Here's how the part is built. I have some questions about the finished solid (model axes, mm). Face numbers are marked on the shaded views. A direction names the side the tool comes from. Coordinates: 2 decimals unless noted, no trailing zeros. Order: outer loops, then holes, each group sorted by start corner. A loop starts at its lowest first (then second) coordinate and runs counter-clockwise, first axis right, second up. Notation, with made-up numbers: M 0.25,39 L 30.25,39 A24 ccw 30.25,71 Z; hole C 0,42.25 d2. An arc over 180 degrees is marked long. One line per question, with ' | ' between items. Start each with the question number.
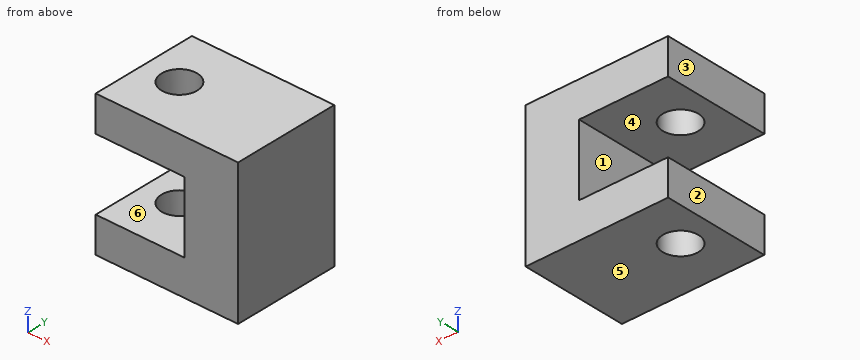
```python
from build123d import *

# Parameters (mm, degrees)
BOSS_EXTRUDE1_DEPTH = 30
SKETCH2_R           = 5
CUT_EXTRUDE1_DEPTH  = 54.851648071


with BuildPart() as part:
    # Sketch1 → Boss-Extrude1 (new body)
    with BuildSketch(Plane(origin=(0, 0, 0), x_dir=(1, 0, 0), z_dir=(0, 1, 0))):
        Polygon((-20, 10), (-20, 20), (20, 20), (20, -20), (-20, -20), (-20, -10), (5, -10), (5, 10), align=None)
    extrude(amount=BOSS_EXTRUDE1_DEPTH)

    # Sketch2 → Cut-Extrude1 (cut, through all)
    with BuildSketch(Plane(origin=(0, 0, -20), x_dir=(-1, 0, 0), z_dir=(0, 0, -1))):
        with Locations((10, 15)):
            Circle(SKETCH2_R)
    extrude(amount=-CUT_EXTRUDE1_DEPTH, mode=Mode.SUBTRACT)


solid = part.part
```
1. I need wall thicknesses on line 1 (Z direction, x = -4, y = 11.75); line 2 (Y direction, x = -10, z = -13.75); line 3 (X direction, y = 25, z = -4). Which ranges of each line are inside material? Lowest first, please.
2. We'd pull the mould along Z, two halves only. Please class the marked faces 3, 4, 5 and 6: released by +Z, released by -Z, zero draft, split by the parting line, or undercut.
3. Imagine slicing it at A-A (x = -10). List the corners of the cut face in (y, z) for me, then the cut area to 3 significant figures.
4. Imagine slicing it at C-C (x = 1.5). List the corners of the cut face in (y, z) for me, then the cut area to 3 significant figures.
5. Imagine slicing it at D-D (y = 25.25). List the corners of the cut face in (x, z) for me, then the cut area to 3 significant figures.
6. Imagine slicing it at B-B (y = 15). List the corners of the cut face in (x, z) for me.
7. Will this pin go through, and if not, where does the flat tip stop? pin 1 (1 mm diameter, centred on y = 24.5, z = -0.5, fed in from -X).
8. Which directions (+Z, -Z, +X, -X, +Y, -Y) give clear straight access to the entire face, cutting with the end or side of a thin tool? Please do the marked faces 1 and 2.
Entries:
1) line 1: -20 to -10, 10 to 20 | line 2: 0 to 10, 20 to 30 | line 3: 5 to 20
2) face 3: zero draft | face 4: undercut | face 5: released by -Z | face 6: undercut
3) outline: M 0,-20 L 10,-20 L 10,-10 L 0,-10 Z; M 0,10 L 10,10 L 10,20 L 0,20 Z; M 20,-20 L 30,-20 L 30,-10 L 20,-10 Z; M 20,10 L 30,10 L 30,20 L 20,20 Z | area: 400 mm²
4) outline: M 0,-20 L 30,-20 L 30,-10 L 0,-10 Z; M 0,10 L 30,10 L 30,20 L 0,20 Z | area: 600 mm²
5) outline: M -20,-20 L 20,-20 L 20,20 L -20,20 L -20,10 L 5,10 L 5,-10 L -20,-10 Z | area: 1,100 mm²
6) outline: M -20,-20 L -15,-20 L -15,-10 L -20,-10 Z; M -20,10 L -15,10 L -15,20 L -20,20 Z; M -5,-20 L 20,-20 L 20,20 L -5,20 L -5,10 L 5,10 L 5,-10 L -5,-10 Z
7) pin 1: x = 5
8) face 1: -X, +Y, -Y | face 2: +Z, -Z, -X, +Y, -Y
